from build123d import *

# Parameters (mm, degrees)
EXTRUDE_962_DEPTH      = 1.25
EXTRUDE_962_DEPTH_BACK = 1.25
SKETCH_1_R             = 1.5


with BuildPart() as part:
    # 草图1 → Extrude 962 (new, two sides: drawn at the far end of the back side and taken through both)
    with BuildSketch(Plane.XY.offset(-EXTRUDE_962_DEPTH_BACK)):
        with BuildLine():
            Line((-11.382159751, -35.030685683), (-13.21047651, -40.657666072))
            ThreePointArc((-13.21047651, -40.657666072), (0, 42.75), (13.21047651, -40.657666072))
            Line((13.21047651, -40.657666072), (11.382159751, -35.030685683))
            ThreePointArc((11.382159751, -35.030685683), (13.598126255, -30.12345555), (18.691961025, -31.868237043))
            ThreePointArc((18.691961025, -31.868237043), (19.991161418, -32.852932397), (21.5917191, -32.543478506))
            ThreePointArc((21.5917191, -32.543478506), (0, 35.95), (-21.5917191, -32.543478506))
            ThreePointArc((-21.5917191, -32.543478506), (-19.991161418, -32.852932397), (-18.691961025, -31.868237043))
            ThreePointArc((-18.691961025, -31.868237043), (-13.598126255, -30.12345555), (-11.382159751, -35.030685683))
        make_face()
        with Locations((-15.388407261, -34.416375782)):
            Circle(SKETCH_1_R, mode=Mode.SUBTRACT)
        with Locations(Location((15.388407261, -34.416375782, 0), (0, 0, 180))):
            Circle(SKETCH_1_R, mode=Mode.SUBTRACT)
    extrude(amount=EXTRUDE_962_DEPTH + EXTRUDE_962_DEPTH_BACK)


solid = part.part
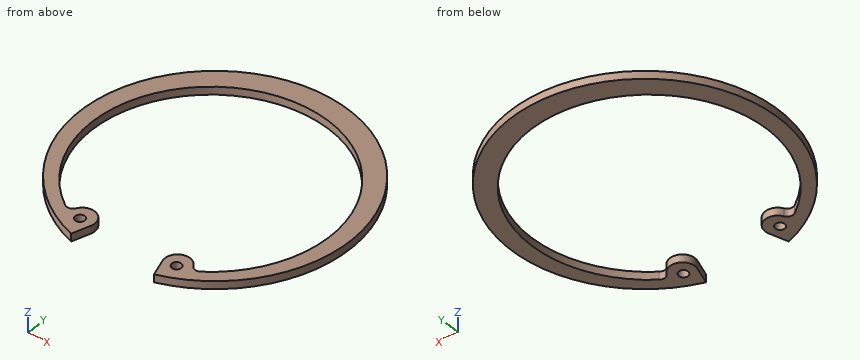
Geometry: final body of the model. Coordinates: model frame, mm. Round coordinates to 2 decimals unless told otherwise and drop trailing zeros. Loops run counter-clockwise (first coordinate to the right, second up) from the corner with the lowest first, then second, coordinate; pieces in that order, holes last.
Q1. Pin query (flat end, axial travel): P1, Ø1, axis at x = -23.5, z = -0.5, coming from the -Y side; P2, Ø1, axis at x = 16.5, z = -0.5, coming from the +Y side. Return the tip coordinate at first contact, or that it passes through.
Q2. Material intervals for L1, parallel to Y at x = -16, z = 0; L2, parallel to Y at x = 0, z = 0.3; L3, parallel to X at y = -7, z = 0.1, sorted ascending.
Q3. Section C-C on x = 0. Return loops of the section in (y, z).
Q4. Section D-D on x = -9.5. Return loops of the section in (y, z), plus the area to 3 significant figures.
Q5. Section A-A on y = 0. Return loops of the section in (x, z), plus the area to 3 significant figures.
Q6. Section B-B on z = 0.75. Return loops of the section in (x, y), plus the area to 3 significant figures.
Evaluation:
1. P1: stops at y = -36.04
1. P2: stops at y = 39.64
2. L1: y = -39.64 to -35.79, -33.05 to -29.88, 32.38 to 39.64
2. L2: y = 35.95 to 42.75
2. L3: x = -42.17 to -37.28, 37.28 to 42.17
3. outline: (35.95, -1.25) - (42.75, -1.25) - (42.75, 1.25) - (35.95, 1.25) - close
4. outline: (34.73, -1.25) - (41.68, -1.25) - (41.68, 1.25) - (34.73, 1.25) - close
4. area: 17.4 mm2
5. outline: (-42.75, -1.25) - (-37.61, -1.25) - (-37.61, 1.25) - (-42.75, 1.25) - close; (37.61, -1.25) - (42.75, -1.25) - (42.75, 1.25) - (37.61, 1.25) - close
5. area: 25.7 mm2
6. outline: (-21.59, -32.54) arc R37.65 cw (long way) to (21.59, -32.54) arc R2 cw to (18.69, -31.87) arc R4 ccw to (11.38, -35.03) - (13.21, -40.66) arc R42.75 ccw (long way) to (-13.21, -40.66) - (-11.38, -35.03) arc R4 ccw to (-18.69, -31.87) arc R2 cw to start; hole circle Ø3 at (-15.39, -34.42); hole circle Ø3 at (15.39, -34.42)
6. area: 1,270 mm2
